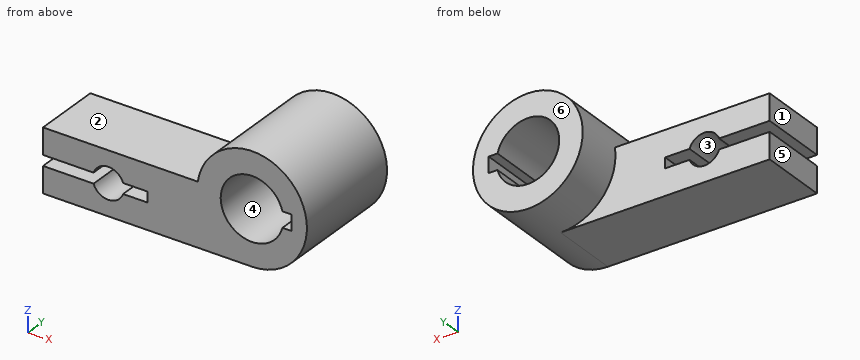
from build123d import *

# Parameters (mm, degrees)
LEVER_ARM_PROFILE_W        = 80
LEVER_ARM_PROFILE_H        = 26
LEVER_ARM_80X26_DEPTH      = 24
HUB_PROFILE_42_R           = 21
HUB_BOSS_42_DEPTH          = 26
HUB_START                  = 18
HUB_EXTENSION_PROFILE_42_R = 21
HUB_EXTENSION_42_DEPTH     = 18
CLAMP_SPLIT_SLOT_DEPTH     = 30
KEYED_BORE_24_DEPTH        = 50


with BuildPart() as part:
    # Lever Arm Profile → Lever Arm 80x26 (new body)
    with BuildSketch(Plane.XY):
        with Locations((40, 13)):
            Rectangle(LEVER_ARM_PROFILE_W, LEVER_ARM_PROFILE_H)
    extrude(amount=-LEVER_ARM_80X26_DEPTH)

    # Hub Profile Ø42 → Hub Boss Ø42 (add)
    with BuildSketch(Plane(origin=(0, 26, 0), x_dir=(1, 0, 0), z_dir=(0, 1, 0))):
        with Locations((80, 3)):
            Circle(HUB_PROFILE_42_R)
    extrude(amount=-HUB_BOSS_42_DEPTH)

    # Hub Extension Profile Ø42 → Hub Extension Ø42 (add)
    with BuildSketch(Plane(origin=(0, 26, 0), x_dir=(1, 0, 0), z_dir=(0, 1, 0)).offset(HUB_START)):
        with Locations(Location((80, 3, 0), (0, 0, 270))):
            Circle(HUB_EXTENSION_PROFILE_42_R)
    extrude(amount=-HUB_EXTENSION_42_DEPTH)

    # Clamp Slot Profile → Clamp Split Slot (cut)
    with BuildSketch(Plane(origin=(0, 26, 0), x_dir=(1, 0, 0), z_dir=(0, 1, 0))):
        with BuildLine():
            Line((0, 14), (0, 10))
            Line((0, 10), (19.343145751, 10))
            ThreePointArc((19.343145751, 10), (25, 6), (30.656854249, 10))
            Line((30.656854249, 10), (40, 10))
            Line((40, 10), (40, 14))
            Line((40, 14), (30.656854249, 14))
            ThreePointArc((30.656854249, 14), (25, 18), (19.343145751, 14))
            Line((19.343145751, 14), (0, 14))
        make_face()
    extrude(amount=-CLAMP_SPLIT_SLOT_DEPTH, mode=Mode.SUBTRACT)

    # Keyed Bore Profile → Keyed Bore Ø24 (cut)
    with BuildSketch(Plane(origin=(0, 44, 0), x_dir=(1, 0, 0), z_dir=(0, 1, 0))):
        with BuildLine():
            Line((95, 6), (91.618950039, 6))
            ThreePointArc((91.618950039, 6), (68, 3), (91.618950039, 0))
            Line((91.618950039, 0), (95, 0))
            Line((95, 0), (95, 6))
        make_face()
    extrude(amount=-KEYED_BORE_24_DEPTH, mode=Mode.SUBTRACT)


solid = part.part
CAD build for the part. Positions are in the model's coordinates, mm. Face numbers are marked on the shaded views. A direction names the side the tool comes from. Round coordinates to 2 decimals unless told otherwise and drop trailing zeros. Write each loop counter-clockwise with the first axis right and the second up, starting at its lowest first coordinate (ties: lowest second). Pieces come first, ordered by that corner, then holes. Notation, with made-up numbers: M 13,-21.75 L 17,-21.75 A29 ccw 17,3.25 Z; hole C -34,10.25 d8. An arc over 180 degrees is marked long. Use a Markdown table: item, result. Add a question column.
1. Slice it at D-D on y = 39.5. Give the cut face in (x, z), then the cut area to 3 significant figures.
2. 3-axis set-ups, long thin cutter, end or side, ignore diameter. For the marked faces 1, 2 and 3: which of +Z, -Z, +X, -X, +Y, -Y reach the whole face in a straight line?
3. Drill centre lines: probe 1 along Z at (x, y) = (80, 23.5); probe 2 along X at (y, z) = (31.5, -3); probe 3 along Y at (x, z) = (56.5, -17). Where is each one in solid material? Low to high.
4. Slice it at B-B on z = -3. Give the cut face in (x, y), then the cut area to 3 significant figures.
5. Pull direction X, two halves, no side cores. Call the marked faces 4, 5 and 6: released by +X, released by -X, zero draft, split by the parting line, or undercut.
6. Slice it at C-C on x = 7. Give the cut face in (y, z), then the cut area to 3 significant figures.
7. Slice it at A-A on y = 14.5. Give the cut face in (x, z).
8. Flat gauge pins, fed straight in: P1, Ø8, axis at y = 23.5, z = -4, coming from the +X side; P2, Ø13, axis at x = 21.5, y = 7, coming from the +Z side; P3, Ø19, axis at x = 52.5, z = -9.5, coming from the +Y side; P4, Ø2, axis at x = 30, z = -7.5, coming from the +Y side. Where does each tip first touch, or does it go through?
Reply:
| question | item | result |
|---|---|---|
| 1 | outline | C 80,-3 d42; hole M 91.62,-6 L 95,-6 L 95,0 L 91.62,0 A12 ccw long Z |
| 1 | area | 914 mm^2 |
| 2 | face 1 | +Z, -Z, -X, +Y, -Y |
| 2 | face 2 | +Z, -X, +Y, -Y |
| 2 | face 3 | +Y, -Y |
| 3 | probe 1 | z = -24 to -15, 9 to 18 |
| 3 | probe 2 | x = 59 to 68, 95 to 101 |
| 3 | probe 3 | y = 0 to 26 |
| 4 | outline | M 0,0 L 68,0 L 68,44 L 59,44 L 59,26 L 0,26 Z; M 95,0 L 101,0 L 101,44 L 95,44 Z |
| 4 | area | 2,190 mm^2 |
| 5 | face 4 | undercut |
| 5 | face 5 | released by -X |
| 5 | face 6 | zero draft |
| 6 | outline | M 0,-24 L 26,-24 L 26,-14 L 0,-14 Z; M 0,-10 L 26,-10 L 26,0 L 0,0 Z |
| 6 | area | 520 mm^2 |
| 7 | outline | M 0,-24 L 80,-24 A21 ccw long 59.22,0 L 0,0 L 0,-10 L 19.34,-10 A6 cw 30.66,-10 L 40,-10 L 40,-14 L 30.66,-14 A6 cw 19.34,-14 L 0,-14 Z; hole M 91.62,-6 L 95,-6 L 95,0 L 91.62,0 A12 ccw long Z |
| 8 | P1 | stops at x = 101 |
| 8 | P2 | stops at z = 0 |
| 8 | P3 | stops at y = 44 |
| 8 | P4 | stops at y = 26 |
